from build123d import *

# Parameters (mm, degrees)
SKETCH_1_W          = 145
SKETCH_1_H          = 55
EXTRUDE_1_DEPTH     = 10
FILLET_1_R          = 8
CUT_EXTRUDE_1_DEPTH = 10


with BuildPart() as part:
    # 草图1 → 凸台-拉伸1 (new body)
    with BuildSketch(Plane.XY):
        Rectangle(SKETCH_1_W, SKETCH_1_H)
    extrude(amount=EXTRUDE_1_DEPTH)

    # 圆角1
    fillet_1_edges = [part.edges().sort_by_distance(p)[0] for p in [
        (72.5, -27.5, 5),
        (-72.5, -27.5, 5),
    ]]
    fillet(fillet_1_edges, radius=FILLET_1_R)

    # 草图2 → 切除-拉伸1 (cut)
    with BuildSketch(Plane.XY.offset(10)):
        with BuildLine():
            Line((51.5, 12), (51.5, -2))
            ThreePointArc((51.5, -2), (46, -7.5), (40.5, -2))
            Line((40.5, -2), (40.5, 12))
            ThreePointArc((40.5, 12), (46, 17.5), (51.5, 12))
        make_face()
        with BuildLine():
            Line((-40.5, 12), (-40.5, -2))
            ThreePointArc((-40.5, -2), (-46, -7.5), (-51.5, -2))
            Line((-51.5, -2), (-51.5, 12))
            ThreePointArc((-51.5, 12), (-46, 17.5), (-40.5, 12))
        make_face()
    extrude(amount=-CUT_EXTRUDE_1_DEPTH, mode=Mode.SUBTRACT)


solid = part.part
Can you work these out from the model? Positions are in its coordinate system, mm. A direction names the side the tool comes from. Give positions to 0.01 mm unless a question says otherwise; leave off trailing zeros. Order: outer loops, then holes, each group sorted by start corner. A loop starts at its lowest first (then second) coordinate and runs counter-clockwise, first axis right, second up. Notation, with made-up numbers: M 12,24 L 62,24 A10 cw 62,37 Z; hole C -34,-2.75 d5. An arc over 180 degrees is marked long. Use a Markdown table: item, result. Add a question column.
Item 1: We'd pull the mould along Y, two halves only. Please class faces 3 (the flat face through (-1, 27.5, 5)), 4 (the flat face through (51.5, 5, 5)), 5 (the cylindrical face through (70.094, -25.219, 5.07)): +Y half, -Y half, draft (parallel to the pull), parting line (faces both ways), or undercut.
Item 2: Suppose I cut it at A-A (y = 1). List the corners of the cut face in (x, z) for me.
Item 3: Suppose I cut it at D-D (x = -45.5). List the corners of the cut face in (y, z) for me.
Item 4: Will this pin go through, and if not, where does the flat tip stop? pin 1 (10 mm diameter, centred on x = 46.5, y = 21, fed in from -Z).
Item 5: Suppose I cut it at B-B (x = 46). List the corners of the cut face in (y, z) for me, then the cut area to 3 significant figures.
Item 6: For faces 1 (the flat face through (-1, 0, 10)), 2 (the cylindrical face through (45.9, 17.5, 5.1)), which set-ups out of +Z, -Z, +X, -X, +Y, -Y let a thin tool reach every point of the face, with its end or its side?
Item 7: If I drill on L1, parallel to X at y = 2, z = 9; L2, parallel to X at y = -3, z = 9; L3, parallel to Y at x = -43.5, z = 5, over which ranges is the centre line in solid material (lowest first)? Write a range as [from, to].
Item 8: Suppose I cut it at C-C (z = 3.25). List the corners of the cut face in (x, y) for me, then the cut area to 3 significant figures.
Answer sheet:
| question | item | result |
|---|---|---|
| 1 | face 3 | +Y half |
| 1 | face 4 | undercut |
| 1 | face 5 | -Y half |
| 2 | outline | M -72.5,0 L -51.5,0 L -51.5,10 L -72.5,10 Z; M -40.5,0 L 40.5,0 L 40.5,10 L -40.5,10 Z; M 51.5,0 L 72.5,0 L 72.5,10 L 51.5,10 Z |
| 3 | outline | M -27.5,0 L -7.48,0 L -7.48,10 L -27.5,10 Z; M 17.48,0 L 27.5,0 L 27.5,10 L 17.48,10 Z |
| 4 | pin 1 | stops at z = 0 |
| 5 | outline | M -27.5,0 L -7.5,0 L -7.5,10 L -27.5,10 Z; M 17.5,0 L 27.5,0 L 27.5,10 L 17.5,10 Z |
| 5 | area | 300 mm² |
| 6 | face 1 | +Z, +X, -X, +Y, -Y |
| 6 | face 2 | +Z, -Z |
| 7 | L1 | x = [-72.5, -51.5], [-40.5, 40.5], [51.5, 72.5] |
| 7 | L2 | x = [-72.5, -51.41], [-40.59, 40.59], [51.41, 72.5] |
| 7 | L3 | y = [-27.5, -6.9], [16.9, 27.5] |
| 8 | outline | M -72.5,-19.5 A8 ccw -64.5,-27.5 L 64.5,-27.5 A8 ccw 72.5,-19.5 L 72.5,27.5 L -72.5,27.5 Z; hole M -51.5,-2 A5.5 ccw -40.5,-2 L -40.5,12 A5.5 ccw -51.5,12 Z; hole M 40.5,-2 A5.5 ccw 51.5,-2 L 51.5,12 A5.5 ccw 40.5,12 Z |
| 8 | area | 7,450 mm² |
